from build123d import *

# Parameters (mm, degrees)
PIVOT_HUB_SKETCH_R           = 15
PIVOT_HUB_30_DEPTH           = 35
BASE_PLATE_DEPTH             = 10
COLUMN_SKETCH_R              = 16
COLUMN_32_DEPTH              = 45
SLOPED_WEB_DEPTH             = 37
WEB_TRIM_CUT_DEPTH           = 37
WEB_PAD_DEPTH                = 17
HUB_CHAMFER_A_SIZE           = 2
HUB_CHAMFER_B_SIZE           = 2
HUB_PIN_HOLE_SKETCH_R        = 2
HUB_PIN_HOLE_4_DEPTH         = 39
COLUMN_TOP_BOSS_SKETCH_R     = 12
COLUMN_TOP_BOSS_24_DEPTH     = 10
TOP_COUNTERBORE_SKETCH_R     = 8
TOP_COUNTERBORE_16_DEPTH     = 3
COLUMN_BORE_SKETCH_R         = 5
COLUMN_BORE_10_DEPTH         = 106
BOTTOM_COUNTERBORE_SKETCH_R  = 6.5
BOTTOM_COUNTERBORE_13_DEPTH  = 7
COLUMN_START                 = -45
COLUMN_SLOT_DEPTH            = 45
BASE_MOUNTING_HOLES_SKETCH_R = 3
BASE_MOUNTING_HOLES_6_DEPTH  = 196


with BuildPart() as part:
    # Pivot Hub Sketch → Pivot Hub Ø30 (new body)
    with BuildSketch(Plane(origin=(0, 0, 0), x_dir=(1, 0, 0), z_dir=(0, 1, 0))):
        with Locations(Location((0, 0, 0), (0, 0, 270))):
            Circle(PIVOT_HUB_SKETCH_R)
    extrude(amount=PIVOT_HUB_30_DEPTH)

    # Base Plate Sketch → Base Plate (add)
    with BuildSketch(Plane(origin=(0, 5, 0), x_dir=(1, 0, 0), z_dir=(0, 1, 0))):
        with BuildLine():
            Line((-94, 0), (-94, 22.5))
            Line((-94, 22.5), (-34, 22.5))
            Line((-34, 22.5), (2.327936287, 14.81825606))
            ThreePointArc((2.327936287, 14.81825606), (-14.994927572, -0.390060375), (3.095195933, -14.677185089))
            Line((3.095195933, -14.677185089), (-34, -22.5))
            Line((-34, -22.5), (-94, -22.5))
            Line((-94, -22.5), (-94, 0))
        make_face()
    extrude(amount=BASE_PLATE_DEPTH)

    # Column Sketch → Column Ø32 (add)
    with BuildSketch(Plane(origin=(0, 15, 0), x_dir=(1, 0, 0), z_dir=(0, 1, 0))):
        with Locations(Location((-74, 0, 0), (0, 0, 90))):
            Circle(COLUMN_SKETCH_R)
    extrude(amount=COLUMN_32_DEPTH)

    # Web Sketch → Sloped Web (add)
    with BuildSketch(Plane(origin=(0, 15, 0), x_dir=(1, 0, 0), z_dir=(0, 1, 0))):
        with BuildLine():
            Line((-74, 11), (-22.154074413, 11))
            ThreePointArc((-22.154074413, 11), (-21, 0), (-22.154074413, -11))
            Line((-22.154074413, -11), (-74, -11))
            ThreePointArc((-74, -11), (-85, 0), (-74, 11))
        make_face()
    extrude(amount=SLOPED_WEB_DEPTH)

    # Web Trim Sketch → Web Trim Cut (cut)
    with BuildSketch(Plane.XY.offset(11)):
        Polygon((-58, 52), (-22.154074413, 52), (-16.501763131, 52), (-16.501763131, 37.711011143), align=None)
    extrude(amount=-WEB_TRIM_CUT_DEPTH, mode=Mode.SUBTRACT)

    # Web Pad Sketch → Web Pad (add)
    with BuildSketch(Plane(origin=(0, 15, 0), x_dir=(1, 0, 0), z_dir=(0, 1, 0))):
        with BuildLine():
            Line((-22.154074413, 11), (-1.869546507, 11))
            Line((-1.869546507, 11), (-1.869546507, -11))
            Line((-1.869546507, -11), (-22.154074413, -11))
            ThreePointArc((-22.154074413, -11), (-21, 0), (-22.154074413, 11))
        make_face()
    extrude(amount=WEB_PAD_DEPTH)

    # Hub Chamfer A
    hub_chamfer_a_edges = [part.edges().sort_by_distance(p)[0] for p in [
        (0, 35, -15),
    ]]
    chamfer(hub_chamfer_a_edges, length=HUB_CHAMFER_A_SIZE)

    # Hub Chamfer B
    hub_chamfer_b_edges = [part.edges().sort_by_distance(p)[0] for p in [
        (0, 0, -15),
    ]]
    chamfer(hub_chamfer_b_edges, length=HUB_CHAMFER_B_SIZE)

    # Hub Pin Hole Sketch → Hub Pin Hole Ø4 (cut)
    with BuildSketch(Plane(origin=(0, 35, 0), x_dir=(1, 0, 0), z_dir=(0, 1, 0))):
        with Locations(Location((0, 0, 0), (0, 0, 270))):
            Circle(HUB_PIN_HOLE_SKETCH_R)
    extrude(amount=-HUB_PIN_HOLE_4_DEPTH, mode=Mode.SUBTRACT)

    # Column Top Boss Sketch → Column Top Boss Ø24 (add)
    with BuildSketch(Plane(origin=(0, 60, 0), x_dir=(1, 0, 0), z_dir=(0, 1, 0))):
        with Locations(Location((-74, 0, 0), (0, 0, 270))):
            Circle(COLUMN_TOP_BOSS_SKETCH_R)
    extrude(amount=COLUMN_TOP_BOSS_24_DEPTH)

    # Top Counterbore Sketch → Top Counterbore Ø16 (cut)
    with BuildSketch(Plane(origin=(0, 70, 0), x_dir=(1, 0, 0), z_dir=(0, 1, 0))):
        with Locations(Location((-74, 0, 0), (0, 0, 270))):
            Circle(TOP_COUNTERBORE_SKETCH_R)
    extrude(amount=-TOP_COUNTERBORE_16_DEPTH, mode=Mode.SUBTRACT)

    # Column Bore Sketch → Column Bore Ø10 (cut)
    with BuildSketch(Plane(origin=(0, 67, 0), x_dir=(1, 0, 0), z_dir=(0, 1, 0))):
        with Locations(Location((-74, 0, 0), (0, 0, 270))):
            Circle(COLUMN_BORE_SKETCH_R)
    extrude(amount=-COLUMN_BORE_10_DEPTH, mode=Mode.SUBTRACT)

    # Bottom Counterbore Sketch → Bottom Counterbore Ø13 (cut)
    with BuildSketch(Plane.XZ.offset(-5)):
        with Locations(Location((-74, 0, 0), (0, 0, 270))):
            Circle(BOTTOM_COUNTERBORE_SKETCH_R)
    extrude(amount=-BOTTOM_COUNTERBORE_13_DEPTH, mode=Mode.SUBTRACT)

    # Column Slot Sketch → Column Slot (cut)
    with BuildSketch(Plane(origin=(0, 60, 0), x_dir=(1, 0, 0), z_dir=(0, 1, 0)).offset(COLUMN_START)):
        with BuildLine():
            ThreePointArc((-62.071178187, 10.663170736), (-66.223257294, 13.982927908), (-71.233832555, 15.759070965))
            Line((-71.233832555, 15.759070965), (-71.233832555, 14.49893024))
            ThreePointArc((-71.233832555, 14.49893024), (-70.680112836, 12.468375582), (-69.172256444, 11))
            ThreePointArc((-69.172256444, 11), (-69.049905074, 10.934960458), (-68.925374416, 10.87419768))
            ThreePointArc((-68.925374416, 10.87419768), (-68.037177922, 10.580431009), (-67.105038845, 10.501004255))
            Line((-67.105038845, 10.501004255), (-62.071178187, 10.663170736))
        make_face()
        with BuildLine():
            Line((-62.071178187, -10.663170736), (-67.105038845, -10.501004255))
            ThreePointArc((-67.105038845, -10.501004255), (-70.016351662, -11.62532842), (-71.233832555, -14.49893024))
            Line((-71.233832555, -14.49893024), (-71.233832555, -15.759070965))
            ThreePointArc((-71.233832555, -15.759070965), (-66.223257294, -13.982927908), (-62.071178187, -10.663170736))
        make_face()
    extrude(amount=COLUMN_SLOT_DEPTH, mode=Mode.SUBTRACT)

    # Base Mounting Holes Sketch → Base Mounting Holes Ø6 (cut)
    with BuildSketch(Plane(origin=(0, 15, 0), x_dir=(1, 0, 0), z_dir=(0, 1, 0))):
        with Locations(Location((-87, -16, 0), (0, 0, 270))):
            Circle(BASE_MOUNTING_HOLES_SKETCH_R)
        with Locations(Location((-62, -16, 0), (0, 0, 270))):
            Circle(BASE_MOUNTING_HOLES_SKETCH_R)
        with Locations(Location((-37, -16, 0), (0, 0, 270))):
            Circle(BASE_MOUNTING_HOLES_SKETCH_R)
        with Locations(Location((-87, 16, 0), (0, 0, 270))):
            Circle(BASE_MOUNTING_HOLES_SKETCH_R)
        with Locations(Location((-37, 16, 0), (0, 0, 270))):
            Circle(BASE_MOUNTING_HOLES_SKETCH_R)
        with Locations(Location((-62, 16, 0), (0, 0, 270))):
            Circle(BASE_MOUNTING_HOLES_SKETCH_R)
    extrude(amount=-BASE_MOUNTING_HOLES_6_DEPTH, mode=Mode.SUBTRACT)


solid = part.part
Here's how the part is built. I have some questions about the finished solid (model axes, mm). A direction names the side the tool comes from. Round coordinates to 2 decimals unless told otherwise and drop trailing zeros. Order: outer loops, then holes, each group sorted by start corner. A loop starts at its lowest first (then second) coordinate and runs counter-clockwise, first axis right, second up. Notation, with made-up numbers: M -8,46 L 18,46 A32 ccw 18,72 Z; hole C -8,2 d7. An arc over 180 degrees is marked long. One line per question, with ' | ' between items.
1) I need wall thicknesses on line 1 (X direction, y = 9.5, z = 0); line 2 (Y direction, x = -18, z = 15); line 3 (Y direction, x = -73, z = -13). Which ranges of each line are inside material? Lowest first, please.
Checked values:
line 1: x = -94 to -80.5, -67.5 to -2, 2 to 15 | line 2: y = 5 to 15 | line 3: y = 5 to 60
2) On a 3-axis mill with a long thin cutter (end or side, diameter ignored), from which of +Z, -Z, +X, -X, +Y, -Y can I reach the whole of each face in a straight line? I mean faces 1 (the cylindrical face through (-66.068, 68.521, -1.041)), 2 (the cylindrical face through (-69.98, 37.18, 11.59)), 3 (the flat face through (-61, 60, 0)), 4 (the flat face through (-59, 52, -8)). Say none if no direction works.
Checked values:
face 1: +Y | face 2: +Z, +Y | face 3: +X, +Y | face 4: -Z, +X, +Y
3) Imagine slicing it at D-D, the plane x = -37. Write out the boundary of the cut face in (y, z).
Checked values:
outline: M 5,-22.5 L 15,-22.5 L 15,-19 L 5,-19 Z; M 5,-13 L 15,-13 L 15,-11 L 44.77,-11 L 44.77,11 L 15,11 L 15,13 L 5,13 Z; M 5,19 L 15,19 L 15,22.5 L 5,22.5 Z
4) Imagine slicing it at C-C, the plane y = 7.5. Count the separate pieces of the cut face and the enclosed holes in it, plus the area to 4 significant figures.
Checked values:
separate pieces: 1 | enclosed holes: 8 | area: 4,025 mm²
5) Imagine slicing it at B-B, the plane x = 0. Write out the boundary of the cut face in (y, z), plus the area to 3 significant figures.
Checked values:
outline: M 0,-13 L 2,-15 L 5,-15 L 5,-15.31 L 15,-15.31 L 15,-15 L 33,-15 L 35,-13 L 35,-2 L 0,-2 Z; M 0,2 L 35,2 L 35,13 L 33,15 L 15,15 L 15,15.33 L 5,15.33 L 5,15 L 2,15 L 0,13 Z | area: 908 mm²
6) I'm going to push flat-ended pins straight in: pin 1 Ø2 at (x, z) = (-59, 4.5) entering from +Y; pin 2 Ø8 at (x, z) = (-62, 16) entering from -Y; pin 3 Ø12 at (y, z) = (44.5, -8.5) entering from -X. Where does each tip first touch, or does it pass through?
Checked values:
pin 1: stops at y = 60 | pin 2: stops at y = 5 | pin 3: stops at x = -89.8
7) Imagine slicing it at A-A, the plane y = 26. Write out the boundary of the cut face in (x, z).
Checked values:
outline: M -71.23,-15.76 L -71.23,-14.5 A4 cw -67.11,-10.5 L -62.07,-10.66 A16 cw -62.38,-11 L -10.2,-11 A15 ccw long -10.2,11 L -62.38,11 A16 cw -62.07,10.66 L -67.11,10.5 A4 cw -71.23,14.5 L -71.23,15.76 A16 ccw long Z; hole C -74,0 d10; hole C 0,0 d4
